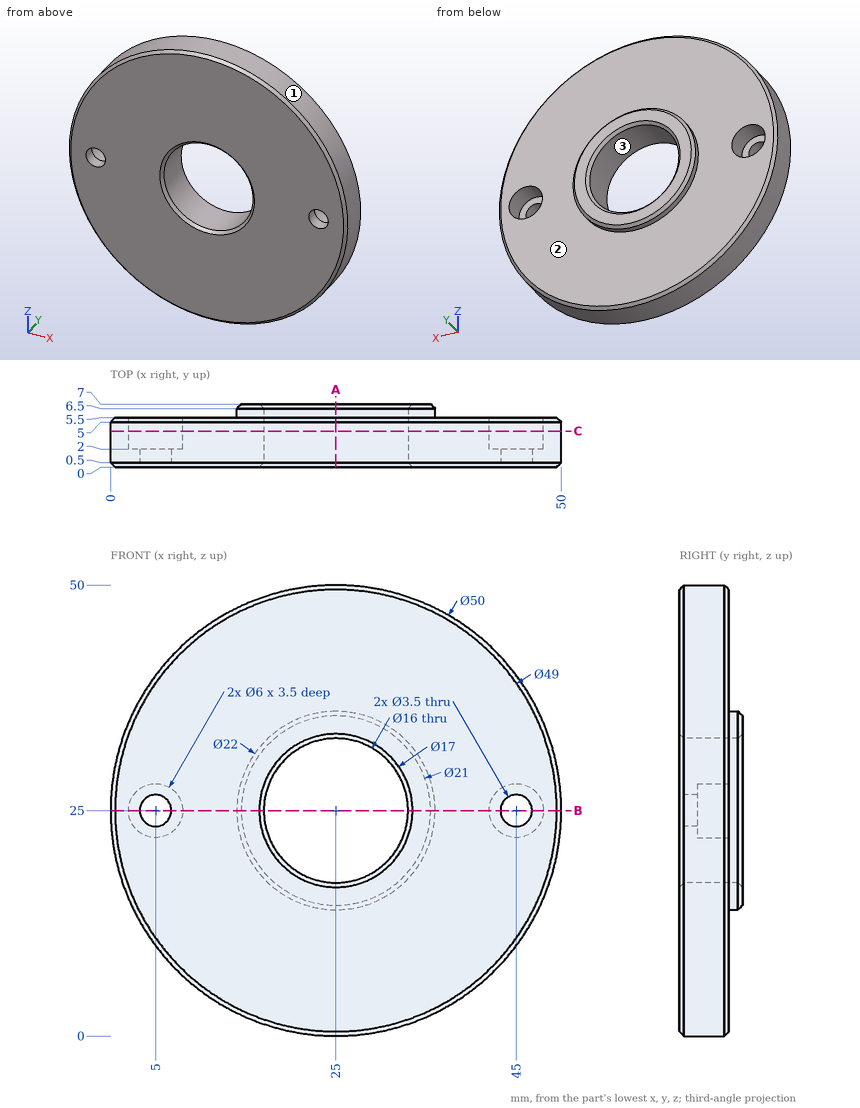
Job drawing, mm, ordinate dimensions from the low corner. One solid piece. Coordinates: 2 decimals unless noted, no trailing zeros. Write each loop counter-clockwise with the first axis right and the second up, starting at its lowest first coordinate (ties: lowest second). Pieces come first, ordered by that corner, then holes. Notation, with made-up numbers: (8.5, 47) -> (52.5, 47) arc R9 ccw to (52.5, 52) -> close; hole circle Ø4 at (14, -13.5). An arc over 180 degrees is marked (long way). Use CSV: the item, a comma, the result in double quotes. Start each with the question number.
Item 1: Band-saw the part on C-C, the plane y = 4. Write the cut outline in (x, z), plus the area to 3 significant figures.
Item 2: Band-saw the part on B-B, the plane z = 25. Give the number of separate pieces and of enclosed holes in the cut face, plus the area to 3 significant figures.
Item 3: Wall check: probe 1 along X at (y, z) = (3.65, 25); probe 2 along X at (y, z) = (0.5, 25); probe 3 along Y at (x, z) = (12.5, 32.5). Give the ranges that are in metal, low to high.
Item 4: Two-plate mould, pull along X, no slides. Class the marked faces 1, 2 and 3: +X half, -X half, draft (parallel to the pull), parting line (faces both ways), or undercut.
Item 5: Drop flat-ended pins along their axis: P1, Ø4, axis at x = 32.5, y = 5.5, coming from the +Z side; P2, Ø1.5, axis at x = 36.5, y = 1, coming from the -Z side; P3, Ø8, axis at x = 45, z = 25, coming from the +Y side. Give the stop position or say it passes through.
Item 6: Band-saw the part on A-A, the plane x = 25. Write the cut outline in (y, z).
Response values:
1,outline,"circle Ø50 at (25, 25); hole circle Ø6 at (5, 25); hole circle Ø16 at (25, 25); hole circle Ø6 at (45, 25)"
1,area,"1,710 mm2"
2,separate pieces,"4"
2,enclosed holes,"0"
2,area,"139 mm2"
3,probe 1,"x = 0 to 2, 8 to 17, 33 to 42, 48 to 50"
3,probe 2,"x = 0 to 3.25, 6.75 to 17, 33 to 43.25, 46.75 to 50"
3,probe 3,"y = 0 to 5.5"
4,face 1,"parting line"
4,face 2,"draft"
4,face 3,"undercut"
5,P1,"stops at z = 49.37"
5,P2,"stops at z = 2.43"
5,P3,"stops at y = 5.5"
6,outline,"(0, 0.5) -> (0.5, 0) -> (5, 0) -> (5.5, 0.5) -> (5.5, 14) -> (6.5, 14) -> (7, 14.5) -> (7, 16.5) -> (6.5, 17) -> (0.5, 17) -> (0, 16.5) -> close; (0, 33.5) -> (0.5, 33) -> (6.5, 33) -> (7, 33.5) -> (7, 35.5) -> (6.5, 36) -> (5.5, 36) -> (5.5, 49.5) -> (5, 50) -> (0.5, 50) -> (0, 49.5) -> close"
